Can you work these out from the drawing? Everything is in mm from the part's minimum corner. Coordinates: 2 decimals unless noted, no trailing zeros. Order: outer loops, then holes, each group sorted by start corner. A loop starts at its lowest first (then second) coordinate and runs counter-clockwise, first axis right, second up. Notation, with made-up numbers: (-27, 63) -> (13, 63) arc R33 ccw to (13, 100) -> close; hole circle Ø5 at (41.25, -33). An arc over 180 degrees is marked (long way). Return JSON: item names as keys, results as strings. Group by question number.
1) If I drill on probe 1 along Y at (x, z) = (6.25, 11.25); probe 2 along Y at (x, z) = (6, 3); probe 3 along Y at (x, z) = (8, 10), over which ranges is the centre line in solid material (lowest first)? Write a range as from..to.
2) If we section it at D-D, the plane z = 1.5: Please give me the cut outline in (x, y), then the cut area to 3 significant figures.
3) Thinking about a two-plate mould opening in Y: for the marked faces 1, 2, 3 and 4, which applies, +Y half, -Y half, draft (parallel to the pull), parting line (faces both ways), or undercut?
4) If we section it at C-C, the plane x = 6: Please give me the cut outline in (y, z).
5) If we section it at A-A, the plane z = 6: Please give me the cut outline in (x, y).
6) For pin 1 (1 mm diameter, centred on x = 10, z = 9, fed in from -Y), with a flat end and sliding along its axis, tell me the tip position at first contact or that it passes through.
7) If we section it at B-B, the plane y = 20: Please give me the cut outline in (x, z).
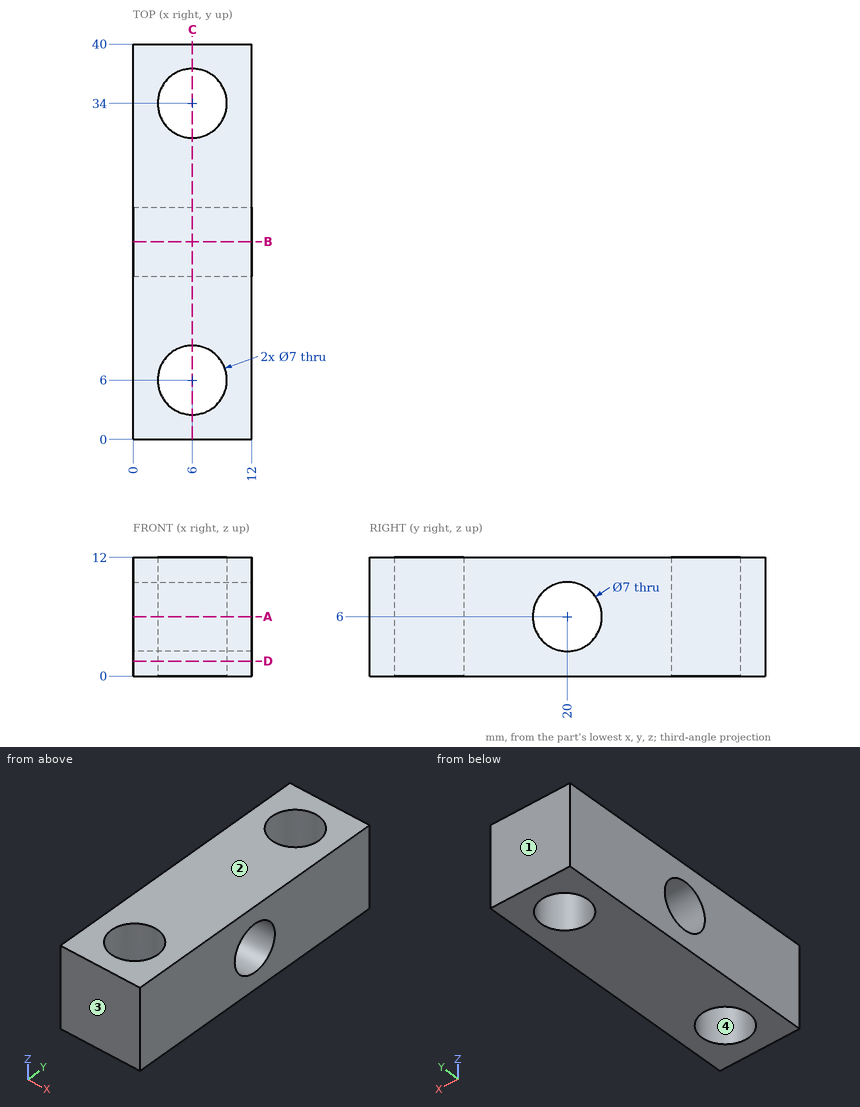
Result sheet:
{
 "1": {"probe 1": "y = 0..2.51, 9.49..30.51, 37.49..40", "probe 2": "y = 0..2.5, 9.5..18.2, 21.8..30.5, 37.5..40", "probe 3": "y = 0..3.13, 8.87..31.13, 36.87..40"},
 "2": {"outline": "(0, 0) -> (12, 0) -> (12, 40) -> (0, 40) -> close; hole circle Ø7 at (6, 6); hole circle Ø7 at (6, 34)", "area": "403 mm2"},
 "3": {"face 1": "+Y half", "face 2": "draft", "face 3": "-Y half", "face 4": "undercut"},
 "4": {"outline": "(0, 0) -> (2.5, 0) -> (2.5, 12) -> (0, 12) -> close; (9.5, 0) -> (30.5, 0) -> (30.5, 12) -> (9.5, 12) -> close; (37.5, 0) -> (40, 0) -> (40, 12) -> (37.5, 12) -> close; hole circle Ø7 at (20, 6)"},
 "5": {"outline": "(0, 0) -> (12, 0) -> (12, 16.5) -> (0, 16.5) -> close; (0, 23.5) -> (12, 23.5) -> (12, 40) -> (0, 40) -> close; hole circle Ø7 at (6, 6); hole circle Ø7 at (6, 34)"},
 "6": {"pin 1": "stops at y = 0"},
 "7": {"outline": "(0, 0) -> (12, 0) -> (12, 2.5) -> (0, 2.5) -> close; (0, 9.5) -> (12, 9.5) -> (12, 12) -> (0, 12) -> close"}
}
